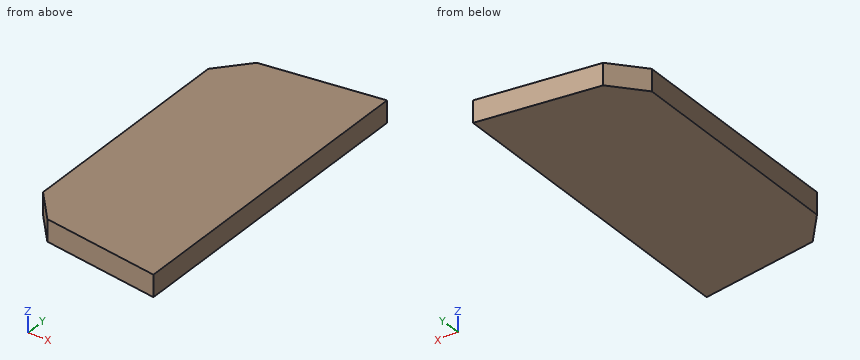
```python
from build123d import *

# Parameters (mm, degrees)
BOSS_EXTRUDE1_DEPTH = 6


with BuildPart() as part:
    # Sketch1 → Boss-Extrude1 (new body)
    with BuildSketch(Plane.XY):
        Polygon((-4, -94.451357529), (-36.682971358, -89.858065454), (-44, -81.440786869), (-44, -18.559213131), (-36.682971358, -10.141934546), (-4, -5.548642471), align=None)
    extrude(amount=BOSS_EXTRUDE1_DEPTH)


solid = part.part
```
Input: part model. Units: mm. Frame: model coordinates. Round coordinates to 2 decimals unless told otherwise and drop trailing zeros. Loops run counter-clockwise (first coordinate to the right, second up) from the corner with the lowest first, then second, coordinate; pieces in that order, holes last. Notation, with made-up numbers: M 77,20 L 122,20 A27 ccw 122,41 Z; hole C -27,-31.5 d9. An arc over 180 degrees is marked long. Answer in a Markdown table with one row per item. Add a question column.
1. Ray query, probe 1 along Y at (x, z) = (-6, 3.85); probe 2 along Y at (x, z) = (-37.5, 4); probe 3 along X at (y, z) = (-14.5, 3.15). Return the intervals inside material, ascending.
2. Section B-B (y = -83). Output: boundary loops of the cut face in (x, z).
3. Contact query for a flat-ended pin moving along its axis: pin 1 (1 mm diameter, centred on x = -19.5, z = 3, fed in from -Y). Output: stop coordinate, or through.
4. Section A-A (z = 5.15). Output: boundary loops of the cut face in (x, y), and give its area (3 significant figures).
5. Section C-C (x = -26.5). Output: boundary loops of the cut face in (y, z), and give its area (3 significant figures).
Values follow:
| question | item | result |
|---|---|---|
| 1 | probe 1 | -94.17 to -5.83 |
| 1 | probe 2 | -88.92 to -11.08 |
| 1 | probe 3 | -40.47 to -4 |
| 2 | outline | M -42.64,0 L -4,0 L -4,6 L -42.64,6 Z |
| 3 | pin 1 | y = -92.34 |
| 4 | outline | M -44,-81.44 L -36.68,-89.86 L -4,-94.45 L -4,-5.55 L -36.68,-10.14 L -44,-18.56 Z |
| 4 | area | 3,280 mm^2 |
| 5 | outline | M -91.29,0 L -8.71,0 L -8.71,6 L -91.29,6 Z |
| 5 | area | 495 mm^2 |
